```python
from build123d import *

# Parameters (mm, degrees)
BOSS_EXTRUDE1_DEPTH = 5
SKETCH4_R           = 0.75
CUT_EXTRUDE1_DEPTH  = 86


with BuildPart() as part:
    # Sketch1 → Boss-Extrude1 (new body)
    with BuildSketch(Plane(origin=(0, 0, 0), x_dir=(1, 0, 0), z_dir=(0, 1, 0))):
        with BuildLine():
            Line((-40, -60), (40, -60))
            ThreePointArc((40, -60), (54.142135624, -54.142135624), (60, -40))
            Line((60, -40), (60, 40))
            ThreePointArc((60, 40), (54.142135624, 54.142135624), (40, 60))
            Line((40, 60), (-40, 60))
            ThreePointArc((-40, 60), (-54.142135624, 54.142135624), (-60, 40))
            Line((-60, 40), (-60, -40))
            ThreePointArc((-60, -40), (-54.142135624, -54.142135624), (-40, -60))
        make_face()
    extrude(amount=BOSS_EXTRUDE1_DEPTH)

    # Sketch4 → Cut-Extrude1 (cut, through all)
    with BuildSketch(Plane(origin=(0, 5, 0), x_dir=(1, 0, 0), z_dir=(0, 1, 0))):
        with Locations(Location((-48, 16.6, 0), (0, 0, 270))):
            Circle(SKETCH4_R)
        with Locations(Location((-28, 16.6, 0), (0, 0, 90))):
            Circle(SKETCH4_R)
        with Locations(Location((-48, 4.6, 0), (0, 0, 90))):
            Circle(SKETCH4_R)
        with Locations(Location((-28, 4.6, 0), (0, 0, 270))):
            Circle(SKETCH4_R)
        with Locations(Location((-28, -4.6, 0), (0, 0, 90))):
            Circle(SKETCH4_R)
        with Locations(Location((-48, -4.6, 0), (0, 0, 270))):
            Circle(SKETCH4_R)
        with Locations(Location((-28, -16.6, 0), (0, 0, 270))):
            Circle(SKETCH4_R)
        with Locations(Location((-48, -16.6, 0), (0, 0, 90))):
            Circle(SKETCH4_R)
        with Locations(Location((28, 41.6, 0), (0, 0, 270))):
            Circle(SKETCH4_R)
        with Locations(Location((48, 41.6, 0), (0, 0, 90))):
            Circle(SKETCH4_R)
        with Locations(Location((28, 29.6, 0), (0, 0, 90))):
            Circle(SKETCH4_R)
        with Locations(Location((48, 29.6, 0), (0, 0, 270))):
            Circle(SKETCH4_R)
        with Locations(Location((48, 8.4, 0), (0, 0, 270))):
            Circle(SKETCH4_R)
        with Locations(Location((28, 8.4, 0), (0, 0, 90))):
            Circle(SKETCH4_R)
        with Locations(Location((28, -8.4, 0), (0, 0, 270))):
            Circle(SKETCH4_R)
        with Locations(Location((48, -8.4, 0), (0, 0, 90))):
            Circle(SKETCH4_R)
        with Locations(Location((28, -20.4, 0), (0, 0, 90))):
            Circle(SKETCH4_R)
        with Locations(Location((48, -20.4, 0), (0, 0, 270))):
            Circle(SKETCH4_R)
        with Locations(Location((48, -29.6, 0), (0, 0, 90))):
            Circle(SKETCH4_R)
        with Locations(Location((28, -29.6, 0), (0, 0, 270))):
            Circle(SKETCH4_R)
        with Locations(Location((48, -41.6, 0), (0, 0, 270))):
            Circle(SKETCH4_R)
        with Locations(Location((28, -41.6, 0), (0, 0, 90))):
            Circle(SKETCH4_R)
    extrude(amount=-CUT_EXTRUDE1_DEPTH, mode=Mode.SUBTRACT)


solid = part.part
```
The listing builds one solid part. Answer for the finished solid, in the listing's coordinates (mm). Give positions to 0.01 mm unless a question says otherwise; leave off trailing zeros. Order: outer loops, then holes, each group sorted by start corner. A loop starts at its lowest first (then second) coordinate and runs counter-clockwise, first axis right, second up. Notation, with made-up numbers: (-9, -14) - (48, -14) arc R5 cw to (48, -5) - close; hole circle Ø10 at (60, 73.25). An arc over 180 degrees is marked (long way). Use one line per item in the form item = value. Start each with the question number.
(1) Flat-ended cylindrical pins translate along their axes: pin 1 Ø1.4 at (x, z) = (48, 29.6) entering from +Y; pin 2 Ø2 at (y, z) = (2.5, -44) entering from -X; pin 3 Ø1.5 at (x, y) = (47.5, 0.5) entering from +Z; pin 4 Ø2 at (y, z) = (1, -45) entering from -X. Find the tip coordinate at first contact, or state that the pin passes through.
(2) A cutting plane is placed at A-A, the plane y = 1.65. State how many separate pieces and enclosed holes the cut face has, then the cut area to 3 significant figures.
(3) A cutting plane is placed at B-B, the plane x = 51. Write down the section's boundary in (y, z).
(4) Consider line 1 (X direction, y = 1.6, z = -8.4); line 2 (X direction, y = 3.45, z = 4.6); line 3 (Z direction, x = -48, y = 3). Determine where each line is inside the solid, lowest interval first. Write a range as from..to.
Ans:
q1.pin_1 = through
q1.pin_2 = -59.77
q1.pin_3 = 58.83
q1.pin_4 = -59.6
q2.separate_pieces = 1
q2.enclosed_holes = 22
q2.area = 14,000 mm^2
q3.outline = (0, -56.7) - (5, -56.7) - (5, 56.7) - (0, 56.7) - close
q4.line_1 = -60..27.25, 28.75..47.25, 48.75..60
q4.line_2 = -60..-48.75, -47.25..-28.75, -27.25..60
q4.line_3 = -58.33..-17.35, -15.85..-5.35, -3.85..3.85, 5.35..15.85, 17.35..58.33
